```python
from build123d import *

# Parameters (mm, degrees)
BOSS_EXTRUDE1_DEPTH = 5
FILLET1_R           = 5
SKETCH2_R           = 3.25
CUT_EXTRUDE1_DEPTH  = 5
BOSS_EXTRUDE2_DEPTH = 5


with BuildPart() as part:
    # Sketch1 → Boss-Extrude1 (new body)
    with BuildSketch(Plane(origin=(0, 210, 0), x_dir=(1, 0, 0), z_dir=(0, 1, 0))):
        with BuildLine():
            Line((-15, 0), (-15, 35))
            Line((-15, 35), (55, 35))
            Line((55, 35), (55, 5))
            Line((55, 5), (14.142135624, 5))
            ThreePointArc((14.142135624, 5), (-2.536529681, 14.783978395), (-15, 0))
        make_face()
    extrude(amount=-BOSS_EXTRUDE1_DEPTH)

    # Fillet1
    fillet1_edges = [part.edges().sort_by_distance(p)[0] for p in [
        (-15, 207.5, -35),
        (55, 207.5, -35),
        (55, 207.5, -5),
    ]]
    fillet(fillet1_edges, radius=FILLET1_R)

    # Sketch2 → Cut-Extrude1 (cut)
    with BuildSketch(Plane(origin=(0, 210, 0), x_dir=(1, 0, 0), z_dir=(0, 1, 0))):
        with Locations(Location((40, 20, 0), (0, 0, 270))):
            Circle(SKETCH2_R)
    extrude(amount=-CUT_EXTRUDE1_DEPTH, mode=Mode.SUBTRACT)

    # Sketch3 → Boss-Extrude2 (add)
    with BuildSketch(Plane(origin=(0, 210, 0), x_dir=(1, 0, 0), z_dir=(0, 1, 0))):
        with BuildLine():
            ThreePointArc((15, 0), (16.464466094, 3.535533906), (20, 5))
            Line((20, 5), (14.142135624, 5))
            ThreePointArc((14.142135624, 5), (14.783978395, 2.536529681), (15, 0))
        make_face()
    extrude(amount=-BOSS_EXTRUDE2_DEPTH)


solid = part.part
```
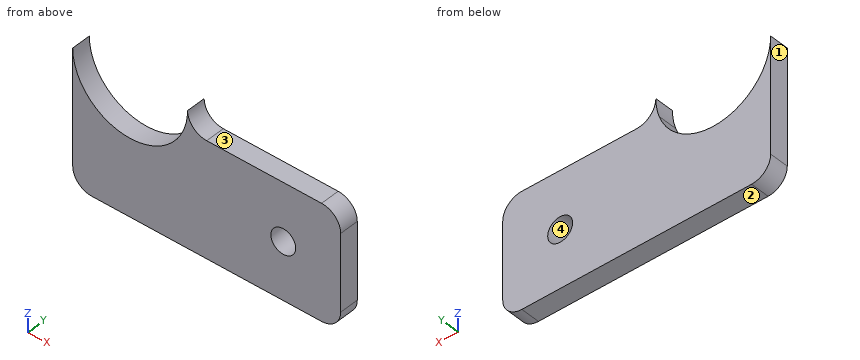
For this review, take the finished solid that the model builds, in its own axes (mm). Face numbers are marked on the shaded views. Round coordinates to 2 decimals unless told otherwise and drop trailing zeros. Write each loop counter-clockwise with the first axis right and the second up, starting at its lowest first coordinate (ties: lowest second). Pieces come first, ordered by that corner, then holes.
1) Take a section at C-C on z = -20. Give the boundary of the cut face in (x, y).
Answer below:
outline: (-15, 205) - (36.75, 205) - (36.75, 210) - (-15, 210) - close; (43.25, 205) - (55, 205) - (55, 210) - (43.25, 210) - close
2) Insertion check: pin 1 Ø1 at (x, y) = (11.5, 205.5) entering from +Z; pin 2 Ø2.5 at (x, y) = (35.5, 207) entering from +Z. Each pin has a flat end and moves straight along its axis. Give the tip position at first contact, or say it passes through.
Answer below:
pin 1: stops at z = -9
pin 2: stops at z = -5
3) Mouldability with a two-part tool opening along Z and no side actions: class the marked faces 1, 2, 3 and 4 as +Z half, -Z half, draft (parallel to the pull), parting line (faces both ways), or undercut.
Answer below:
face 1: draft
face 2: -Z half
face 3: +Z half
face 4: undercut
4) For line 1 along X through (y, z) = (206, -20); line 2 along X through (y, z) = (207.55, -3.5); line 3 along Z through (x, y) = (38, 207.5), list the stretches that pass through material, from the lowest coordinate up.
Answer below:
line 1: x = -15 to 36.75, 43.25 to 55
line 2: x = -15 to -14.59, 14.59 to 16.43
line 3: z = -35 to -22.56, -17.44 to -5
5) Take a section at B-B on y = 206.4. Give the boundary of the cut face in (x, z).
Answer below:
outline: (-15, -30) arc R5 ccw to (-10, -35) - (50, -35) arc R5 ccw to (55, -30) - (55, -10) arc R5 ccw to (50, -5) - (20, -5) arc R5 cw to (15, 0) arc R15 cw to (-15, 0) - close; hole circle Ø6.5 at (40, -20)
6) Take a section at A-A on x = 40. Give the boundary of the cut face in (y, z), then the cut area to 4 significant figures.
Answer below:
outline: (205, -35) - (210, -35) - (210, -23.25) - (205, -23.25) - close; (205, -16.75) - (210, -16.75) - (210, -5) - (205, -5) - close
area: 117.5 mm2
7) Take a section at D-D on x = 48. Give the boundary of the cut face in (y, z), then the cut area to 3 significant figures.
Answer below:
outline: (205, -35) - (210, -35) - (210, -5) - (205, -5) - close
area: 150 mm2
